Here's the drawing with two shaded views (mm, measured from the low corner). I have some questions. A direction names the side the tool comes from. Round coordinates to 2 decimals unless told otherwise and drop trailing zeros. Order: outer loops, then holes, each group sorted by start corner. A loop starts at its lowest first (then second) coordinate and runs counter-clockwise, first axis right, second up.
Q1. If we section it at A-A (x = 87.5): Count the separate pieces of the cut face and the enclosed holes in it, plus the area to 3 significant figures.
Q2. We'd pull the mould along Z, two halves only. Please class the marked faces 3, 4 and 5: pulls with the +Z half, pulls with the -Z half, needs draft (parallel to the pull), parting line crosses it, or undercut.
Q3. If I drill on line 1 (Z direction, x = 25.5, y = 38); line 2 (X direction, y = 1, z = 30), over which ranges is the centre line in solid material (lowest first)?
Q4. If we section it at B-B (y = 15): Please give me the cut outline in (x, z), plus the area to 3 significant figures.
Q5. If we section it at D-D (x = 353): Please give me the cut outline in (y, z), plus the area to 3 significant figures.
Q6. For the marked faces 1 and 2, which set-ups out of +Z, -Z, +X, -X, +Y, -Y let a thin tool reach every point of the face, with its end or its side?
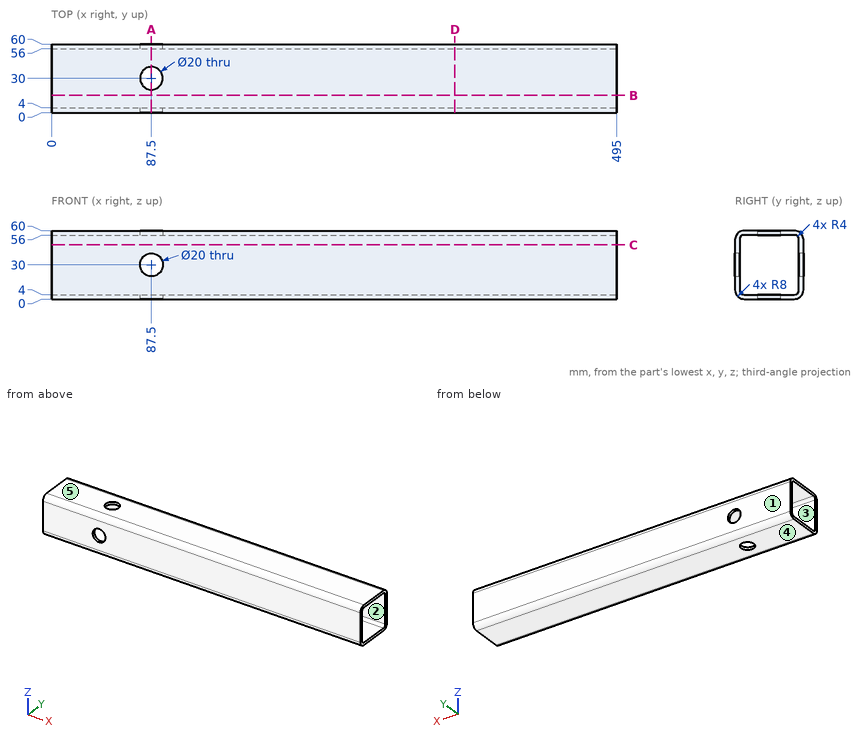
Solution:
1. separate pieces: 4
1. enclosed holes: 0
1. area: 535 mm2
2. face 3: undercut
2. face 4: pulls with the -Z half
2. face 5: pulls with the +Z half
3. line 1: z = 0 to 4, 56 to 60
3. line 2: x = 0 to 77.5, 97.5 to 495
4. outline: (0, 0) - (495, 0) - (495, 4) - (0, 4) - close; (0, 56) - (495, 56) - (495, 60) - (0, 60) - close
4. area: 3,960 mm2
5. outline: (0, 8) arc R8 ccw to (8, 0) - (52, 0) arc R8 ccw to (60, 8) - (60, 52) arc R8 ccw to (52, 60) - (8, 60) arc R8 ccw to (0, 52) - close; hole (4, 8) arc R4 ccw to (8, 4) - (52, 4) arc R4 ccw to (56, 8) - (56, 52) arc R4 ccw to (52, 56) - (8, 56) arc R4 ccw to (4, 52) - close
5. area: 855 mm2
6. face 1: +Z, -Z, +X, -X, +Y
6. face 2: +X, -X
